Geometry check sheet. Reference: the model listing, model coordinates, mm. Round coordinates to 2 decimals unless told otherwise and drop trailing zeros. Order: outer loops, then holes, each group sorted by start corner. A loop starts at its lowest first (then second) coordinate and runs counter-clockwise, first axis right, second up. Notation, with made-up numbers: (85, -27.75) - (137, -27.75) arc R27 ccw to (137, 6.25) - close; hole circle Ø6 at (15, 41.25). An arc over 180 degrees is marked (long way). Use a Markdown table: item, result. Add a question column.
(1) Mould release check, pull along Z, two halves, no side actions. Record for faces 1 (the face through (-12.932, 1.96, 5.362)), 2 (the face through (-10, 5, 12)), 3 (the face through (0, 2, -18)): released by +Z, released by -Z, zero draft, split by the parting line, or undercut.
(2) Thickness scan on line 1 along Z through (x, y) = (0, 3.15); line 2 along Z through (x, y) = (-12, 1.05); line 3 along X through (y, z) = (1.7, -10). Record the ranges inside material, lowest first. Write a range as [from, to].
(3) Section check B-B on y = 2. Record the boundary of the cut face in (x, z).
(4) Section check A-A on x = 0. Record the boundary of the cut face in (y, z) (3 decimals), then the cut area to 3 significant figures.
(5) Gauge pin test, flat ends, axial feed: P1, Ø2, axis at y = 3.5, z = -8.5, coming from the +X side; P2, Ø3, axis at y = 2, z = -9.5, coming from the -X side. Record the tip position at first contact, or that the pin passes through.
```python
from build123d import *

# Parameters (mm, degrees)
BOSS_EXTRUDE1_DEPTH              = 5
M30X2_0_TAPPED_HOLE1_D           = 28
M30X2_0_TAPPED_HOLE1_DEPTH       = 70
M30X2_0_TAPPED_HOLE1_CSINK_D     = 30.05
M30X2_0_TAPPED_HOLE1_CSINK_ANGLE = 90
M30X2_0_TAPPED_HOLE1_TIP         = 8.412048666


with BuildPart() as part:
    # Sketch1 → Boss-Extrude1 (new body)
    with BuildSketch(Plane(origin=(0, 0, 0), x_dir=(1, 0, 0), z_dir=(0, 1, 0))):
        with BuildLine():
            Line((10.816653826, 18), (-10.816653826, 18))
            ThreePointArc((-10.816653826, 18), (-21, 0), (-10.816653826, -18))
            Line((-10.816653826, -18), (10.816653826, -18))
            ThreePointArc((10.816653826, -18), (18.277714988, -10.340461055), (21, 0))
            ThreePointArc((21, 0), (18.277714988, 10.340461055), (10.816653826, 18))
        make_face()
    extrude(amount=BOSS_EXTRUDE1_DEPTH)

    # M30x2.0 Tapped Hole1
    with Locations(Plane(origin=(0, 5, 0), x_dir=(1, 0, 0), z_dir=(0, 1, 0))):
        with Locations((0, 0)):
            CounterSinkHole(M30X2_0_TAPPED_HOLE1_D / 2, M30X2_0_TAPPED_HOLE1_CSINK_D / 2, depth=M30X2_0_TAPPED_HOLE1_DEPTH, counter_sink_angle=M30X2_0_TAPPED_HOLE1_CSINK_ANGLE)
            with Locations((0, 0, -(M30X2_0_TAPPED_HOLE1_DEPTH + M30X2_0_TAPPED_HOLE1_TIP / 2))):  # 118° drill point
                Cone(0, M30X2_0_TAPPED_HOLE1_D / 2, M30X2_0_TAPPED_HOLE1_TIP, mode=Mode.SUBTRACT)


solid = part.part
```
Check sheet entries:
| question | item | result |
|---|---|---|
| 1 | face 1 | undercut |
| 1 | face 2 | zero draft |
| 1 | face 3 | released by -Z |
| 2 | line 1 | z = [-18, -14], [14, 18] |
| 2 | line 2 | z = [-17.23, -7.21], [7.21, 17.23] |
| 2 | line 3 | x = [-18.47, -9.8], [9.8, 18.47] |
| 3 | outline | (-10.82, -18) - (10.82, -18) arc R21 ccw to (10.82, 18) - (-10.82, 18) arc R21 ccw to start; hole circle Ø28 at (0, 0) |
| 4 | outline | (0, -18) - (5, -18) - (5, -15.025) - (3.975, -14) - (0, -14) - close; (0, 14) - (3.975, 14) - (5, 15.025) - (5, 18) - (0, 18) - close |
| 4 | area | 38.9 mm2 |
| 5 | P1 | stops at x = 19.62 |
| 5 | P2 | stops at x = -19.42 |
